```python
from build123d import *

# Parameters (mm, degrees)
EXTRUDE_1_DEPTH     = 20
FILLET_1_R          = 1
SKETCH_2_R          = 3
CUT_EXTRUDE_1_DEPTH = 78.356318423


with BuildPart() as part:
    # 草图1 → 凸台-拉伸1 (new body)
    with BuildSketch(Plane.XY):
        with BuildLine():
            Line((0, 0), (15, 0))
            Line((15, 0), (15, 20))
            Line((15, 20), (57, 20))
            Line((57, 20), (57, 0))
            Line((57, 0), (72, 0))
            Line((72, 0), (72, -9.5))
            Line((72, -9.5), (50.5, -9.5))
            Line((50.5, -9.5), (50.5, 0))
            ThreePointArc((50.5, 0), (36, 14.5), (21.5, 0))
            Line((21.5, 0), (21.5, -9.5))
            Line((21.5, -9.5), (0, -9.5))
            Line((0, -9.5), (0, 0))
        make_face()
    extrude(amount=EXTRUDE_1_DEPTH)

    # 圆角1
    fillet_1_edges = [part.edges().sort_by_distance(p)[0] for p in [
        (15, 20, 10),
        (57, 20, 10),
    ]]
    fillet(fillet_1_edges, radius=FILLET_1_R)

    # 草图2 → 切除-拉伸1 (cut, through all)
    with BuildSketch(Plane(origin=(0, 0, 0), x_dir=(1, 0, 0), z_dir=(0, 1, 0))):
        with Locations(Location((6.5, -10, 0), (0, 0, 270))):
            Circle(SKETCH_2_R)
        with Locations(Location((66.5, -10, 0), (0, 0, 270))):
            Circle(SKETCH_2_R)
    extrude(amount=-CUT_EXTRUDE_1_DEPTH, mode=Mode.SUBTRACT)


solid = part.part
```
CAD build for the part. Positions are in the model's coordinates, mm. A direction names the side the tool comes from. Give positions to 0.01 mm unless a question says otherwise; leave off trailing zeros. Write each loop counter-clockwise with the first axis right and the second up, starting at its lowest first coordinate (ties: lowest second). Pieces come first, ordered by that corner, then holes. Notation, with made-up numbers: M 77,-16 L 116,-16 A20 cw 116,3 Z; hole C 26,-23 d8. An arc over 180 degrees is marked long. Return JSON: item names as keys, results as strings. Group by question number.
(1) Mould opens along Y. For faces 4 (the face through (9, 0, 8)), 5 (the face through (11, -9.5, 10)), 6 (the face through (15, 9, 10)) say: pulls with the +Y half, pulls with the -Y half, needs draft (parallel to the pull), parting line crosses it, or undercut.
(2) Band-saw the part on B-B (z = 10). Give the cut face in (x, y), and give its area (3 significant figures).
(3) Band-saw the part on C-C (x = 66.5). Give the cut face in (y, z).
(4) Drill centre lines: L1, parallel to X at y = -3.5, z = 10; L2, parallel to X at y = -6, z = 6.75; L3, parallel to Y at x = 60, z = 6.75. Where is each one in solid material? Low to high. Write a range as [from, to].
(5) 3-axis set-ups, long thin cutter, end or side, ignore diameter. For faces 1 (the face through (63, 0, 10)), 2 (the face through (50.5, -5, 10)), 3 (the face through (63.57, -4.68, 9.35)): which of +Z, -Z, +X, -X, +Y, -Y reach the whole face in a straight line?
(6) Band-saw the part on D-D (y = 9.5). Give the cut face in (x, z), and give its area (3 significant figures).
(7) Band-saw the part on A-A (y = -6). Give the cut face in (x, z).
(8) Flat gauge pins, fed straight in: pin 1 Ø8 at (x, z) = (66.5, 10) entering from +Y; pin 2 Ø4 at (y, z) = (17, 17) entering from +X; pin 3 Ø7 at (x, z) = (6.5, 10) entering from -Y; pin 4 Ø5.5 at (y, z) = (9.5, 10) entering from -X. Where does each tip first touch, or does it go through?
Entries:
{
 "1": {"face 4": "pulls with the +Y half", "face 5": "pulls with the -Y half", "face 6": "needs draft"},
 "2": {"outline": "M 0,-9.5 L 3.5,-9.5 L 3.5,0 L 0,0 Z; M 9.5,-9.5 L 21.5,-9.5 L 21.5,0 A14.5 cw 50.5,0 L 50.5,-9.5 L 63.5,-9.5 L 63.5,0 L 57,0 L 57,19 A1 ccw 56,20 L 16,20 A1 ccw 15,19 L 15,0 L 9.5,0 Z; M 69.5,-9.5 L 72,-9.5 L 72,0 L 69.5,0 Z", "area": "804 mm^2"},
 "3": {"outline": "M -9.5,0 L 0,0 L 0,7 L -9.5,7 Z; M -9.5,13 L 0,13 L 0,20 L -9.5,20 Z"},
 "4": {"L1": "x = [0, 3.5], [9.5, 21.5], [50.5, 63.5], [69.5, 72]", "L2": "x = [0, 21.5], [50.5, 72]", "L3": "y = [-9.5, 0]"},
 "5": {"face 1": "+Z, -Z, +X, +Y", "face 2": "+Z, -Z, -Y", "face 3": "+Y, -Y"},
 "6": {"outline": "M 15,0 L 25.05,0 L 25.05,20 L 15,20 Z; M 46.95,0 L 57,0 L 57,20 L 46.95,20 Z", "area": "402 mm^2"},
 "7": {"outline": "M 0,0 L 21.5,0 L 21.5,20 L 0,20 Z; M 50.5,0 L 72,0 L 72,20 L 50.5,20 Z; hole C 6.5,10 d6; hole C 66.5,10 d6"},
 "8": {"pin 1": "stops at y = 0", "pin 2": "stops at x = 57", "pin 3": "stops at y = -9.5", "pin 4": "stops at x = 15"}
}
